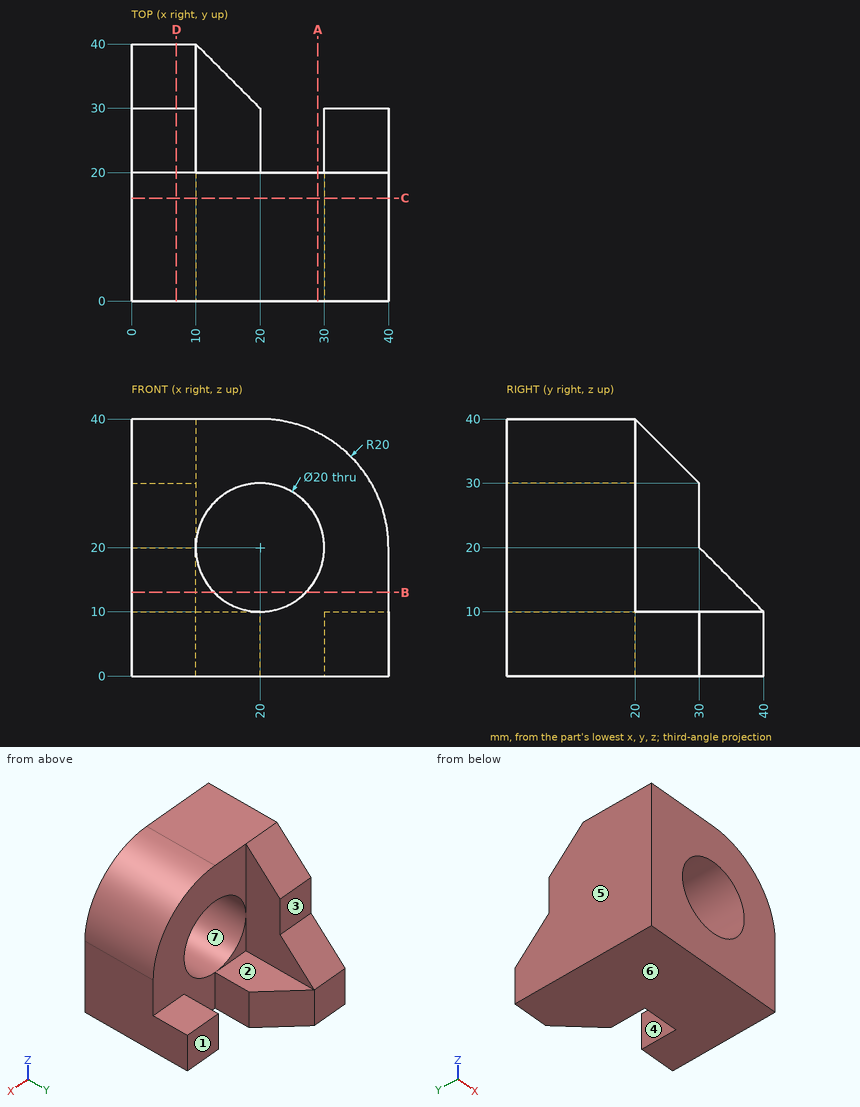
Here's the drawing with two shaded views (mm, measured from the low corner). I have some questions. A direction names the side the tool comes from. Give positions to 0.01 mm unless a question says otherwise; leave off trailing zeros. Loops run counter-clockwise (first coordinate to the right, second up) from the corner with the lowest first, then second, coordinate; pieces in that order, holes last. Notation, with made-up numbers: M 81,54 L 122,54 A18 ccw 122,78 Z; hole C 11,-8.75 d5. An arc over 180 degrees is marked long. One line per item, written item: value. Start each with the question number.
1) If we section it at A-A, the plane x = 29: Write out the boundary of the cut face in (y, z).
2) If we section it at C-C, the plane y = 16: Write out the boundary of the cut face in (x, z), and give its area (3 significant figures).
3) On a 3-axis mill with a long thin cutter (end or side, diameter ignored), from which of +Z, -Z, +X, -X, +Y, -Y can I reach the whole of each face in a straight line? I mean the marked faces 1, 2, 3 and 4. Say none if no direction works.
4) I'm going to push flat-ended pins straight in: pin 1 (1.5 mm diameter, centred on x = 32.5, z = 10, fed in from +Y); pin 2 (12 mm diameter, centred on x = 10.5, y = 27, fed in from +Z); pin 3 (3 mm diameter, centred on y = 9, z = 31, fed in from +X); pin 4 (12 mm diameter, centred on x = 22.5, z = 18.5, fed in from -Y). Where does each tip first touch, or does it pass through?
5) If we section it at D-D, the plane x = 7: Write out the boundary of the cut face in (y, z), and give its area (3 significant figures).
6) Thinking about a two-plate mould opening in X: for the marked faces 5, 6 and 7, which applies, +X half, -X half, draft (parallel to the pull), parting line (faces both ways), or undercut?
7) If we section it at B-B, the plane z = 13: Write out the boundary of the cut face in (x, y).
8) If I drill on line 1 (Z direction, x = 20, y = 11); line 2 (Y direction, x = 32.5, z = 8), over which ranges is the centre line in solid material (lowest first)? Write a range as [from, to].
Completed:
1. outline: M 0,0 L 20,0 L 20,15.64 L 0,15.64 Z; M 0,24.36 L 20,24.36 L 20,37.86 L 0,37.86 Z
2. outline: M 0,0 L 40,0 L 40,20 A20 ccw 20,40 L 0,40 Z; hole C 20,20 d20
2. area: 1,200 mm^2
3. face 1: +Z, -Z, +X, +Y
3. face 2: +Z, +X, +Y
3. face 3: +Z, +X, -X, +Y
3. face 4: +Z, -Z, +Y
4. pin 1: stops at y = 30
4. pin 2: stops at z = 38.98
4. pin 3: stops at x = 37.6
4. pin 4: passes through
5. outline: M 0,0 L 40,0 L 40,10 L 30,20 L 30,30 L 20,40 L 0,40 Z
5. area: 1,300 mm^2
6. face 5: -X half
6. face 6: draft
6. face 7: undercut
7. outline: M 0,0 L 12.86,0 L 12.86,20 L 10,20 L 10,37 L 0,37 Z; M 27.14,0 L 40,0 L 40,20 L 27.14,20 Z
8. line 1: z = [0, 10], [30, 40]
8. line 2: y = [0, 30]
